```python
from build123d import *

# Parameters (mm, degrees)
BOSS_EXTRUDE1_DEPTH = 14
FILLET1_R           = 0.8


with BuildPart() as part:
    # Sketch1 → Boss-Extrude1 (new body)
    with BuildSketch(Plane.XY):
        with BuildLine():
            Line((-67.5, 11), (67.5, 11))
            ThreePointArc((67.5, 11), (78.5, 0), (67.5, -11))
            Line((67.5, -11), (-67.5, -11))
            ThreePointArc((-67.5, -11), (-78.5, 0), (-67.5, 11))
        make_face()
    extrude(amount=BOSS_EXTRUDE1_DEPTH)

    # Fillet1
    fillet1_edges = [part.edges().sort_by_distance(p)[0] for p in [
        (78.5, 0, 14),
        (0, 11, 14),
        (-78.5, 0, 14),
        (0, 11, 0),
        (78.5, 0, 0),
        (0, -11, 0),
        (-78.5, 0, 0),
        (0, -11, 14),
    ]]
    fillet(fillet1_edges, radius=FILLET1_R)


solid = part.part
```
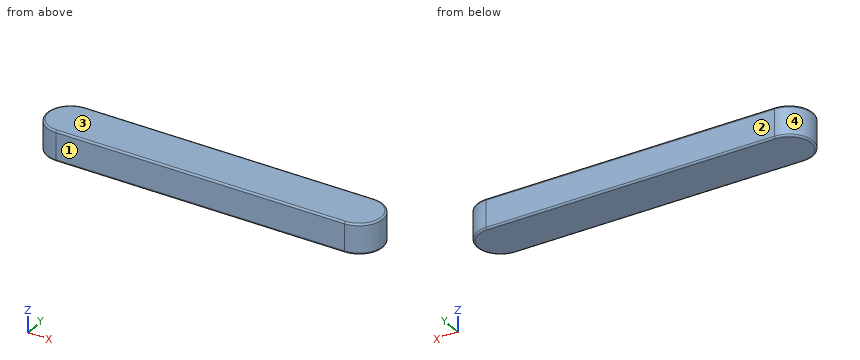
Could you check a few things on this model? Use its own coordinates, in mm. Face numbers are marked on the shaded views. Round coordinates to 2 decimals unless told otherwise and drop trailing zeros. Write each loop counter-clockwise with the first axis right and the second up, starting at its lowest first coordinate (ties: lowest second). Pieces come first, ordered by that corner, then holes.
(1) If I drill on probe 1 along X at (y, z) = (-0.5, 11.75); probe 2 along X at (y, z) = (9.5, 3), over which ranges is the centre line in solid material (lowest first)?
Findings below:
probe 1: x = -78.49 to 78.49
probe 2: x = -73.05 to 73.05
(2) Suppose I cut it at A-A on z = 9. Write out the boundary of the cut face in (x, y).
Findings below:
outline: (-67.5, -11) - (67.5, -11) arc R11 ccw to (67.5, 11) - (-67.5, 11) arc R11 ccw to start
(3) Thinking about a two-plate mould opening in Y: for the marked faces 1, 2, 3 and 4, which applies, +Y half, -Y half, draft (parallel to the pull), parting line (faces both ways), or undercut?
Findings below:
face 1: -Y half
face 2: +Y half
face 3: draft
face 4: parting line
